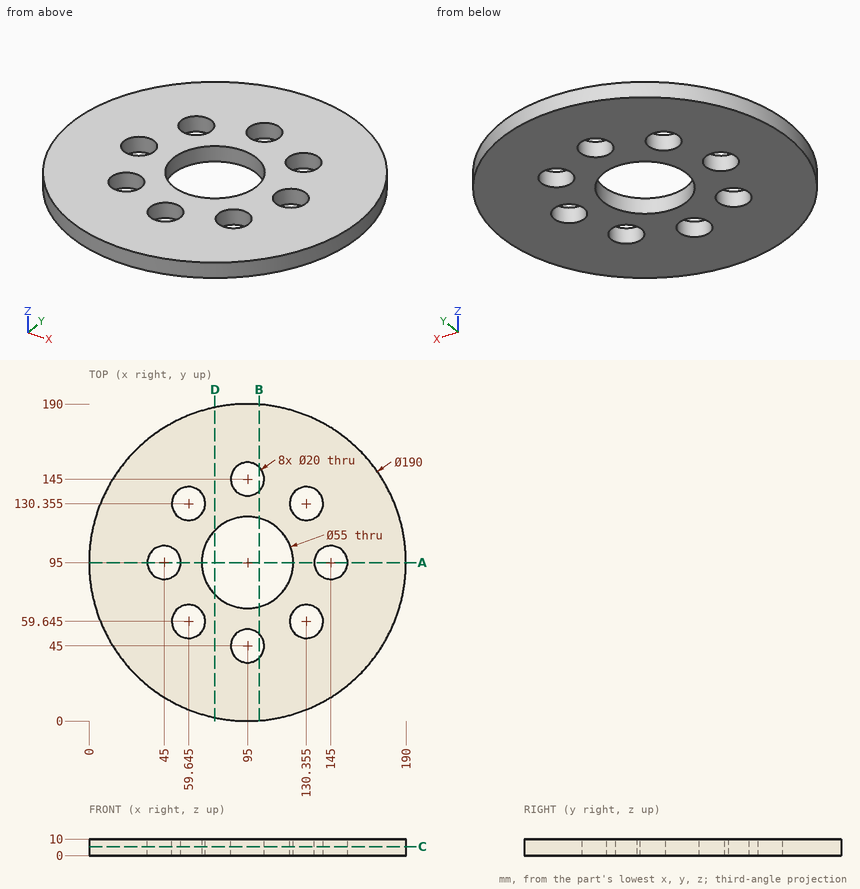
For this review, use the dimensioned drawing (mm, ordinates from the lowest corner) and the shaded views. Coordinates: 2 decimals unless noted, no trailing zeros. Order: outer loops, then holes, each group sorted by start corner. A loop starts at its lowest first (then second) coordinate and runs counter-clockwise, first axis right, second up. Notation, with made-up numbers: M 4,75.25 L 32,75.25 A30 cw 32,98.25 Z; hole C 88.5,24.5 d10. An arc over 180 degrees is marked long. Answer as a JSON object with one key per item and string values. Group by question number.
1) Add section A-A, the plane y = 95. Write out the cut boundary in (x, z), then the cut area to 3 significant figures.
2) For pin 1 (4 mm diameter, centred on x = 162.5, y = 113, fed in from -Z); pin 2 (6 mm diameter, centred on x = 161, z = 4, fed in from -Y) (1 decimal); pin 3 (3 mm diameter, centred on y = 107, z = 8, fed in from -X); pin 4 (3 mm diameter, centred on x = 116, z = 1, fed in from -Y), all flat-tipped, find the tip position at first contact; note any pin that passes through.
3) Add section B-B, the plane x = 102. Write out the cut boundary in (y, z), then the cut area to 3 significant figures.
4) Add section C-C, the plane z = 5.5. Count the separate pieces of the cut face and the enclosed holes in it, then the cut area to 3 significant figures.
5) Add section D-D, the plane x = 75.5. Write out the cut boundary in (y, z), then the cut area to 3 significant figures.
6) Wall thickness on L1, parallel to Y at x = 125.5, z = 3.5; L2, parallel to Y at x = 87, z = 3.25 (1 decimal); L3, parallel to X at y = 89.5, z = 8.75 (1 decimal): over which ranges is each line inside the solid? List them lowest first.
Computed values:
{
 "1": {"outline": "M 0,0 L 35,0 L 35,10 L 0,10 Z; M 55,0 L 67.5,0 L 67.5,10 L 55,10 Z; M 122.5,0 L 135,0 L 135,10 L 122.5,10 Z; M 155,0 L 190,0 L 190,10 L 155,10 Z", "area": "950 mm^2"},
 "2": {"pin 1": "stops at z = 0", "pin 2": "stops at y = 23.9", "pin 3": "stops at x = 0.58", "pin 4": "stops at y = 2.02"},
 "3": {"outline": "M 0.26,0 L 37.86,0 L 37.86,10 L 0.26,10 Z; M 52.14,0 L 68.41,0 L 68.41,10 L 52.14,10 Z; M 121.59,0 L 137.86,0 L 137.86,10 L 121.59,10 Z; M 152.14,0 L 189.74,0 L 189.74,10 L 152.14,10 Z", "area": "1,080 mm^2"},
 "4": {"separate pieces": "1", "enclosed holes": "9", "area": "23,500 mm^2"},
 "5": {"outline": "M 2.02,0 L 75.61,0 L 75.61,10 L 2.02,10 Z; M 114.39,0 L 187.98,0 L 187.98,10 L 114.39,10 Z", "area": "1,470 mm^2"},
 "6": {"L1": "y = 5.03 to 50.9, 68.39 to 121.61, 139.1 to 184.97", "L2": "y = 0.3 to 39, 51 to 68.7, 121.3 to 139, 151 to 189.7", "L3": "x = 0.2 to 36.6, 53.4 to 68.1, 121.9 to 136.6, 153.4 to 189.8"}
}
